Verification items for the finished model (mm, model axes). A direction names the side the tool comes from. Give positions to 0.01 mm unless a question says otherwise; leave off trailing zeros. Write each loop counter-clockwise with the first axis right and the second up, starting at its lowest first coordinate (ties: lowest second). Pieces come first, ordered by that corner, then holes. Notation, with made-up numbers: (39.25, 82.5) - (90.25, 82.5) arc R16 ccw to (90.25, 87.5) - close; hole circle Ø9 at (23.25, -24). An arc over 180 degrees is marked (long way). Answer as a JSON object with one key per item and string values. Group by question number.
Item 1: Scan lines: line 1 along X through (y, z) = (20, 0); line 2 along X through (y, z) = (37.5, -1); line 3 along Z through (x, y) = (70, 28.5). Record each from-to range of solid material in increasing order. Write a range as [from, to].
Item 2: Sectioned sample at B-B, the plane z = 0. Record the boundary of the cut face in (x, y).
Item 3: Sectioned sample at D-D, the plane z = 143. Record the boundary of the cut face in (x, y), and give its area (3 significant figures).
Item 4: Tool access check on faces 1 (the face through (112.81, 27.54, 63.11)), 2 (the face through (31, 40, 52)), 3 (the face through (-2, 25, -122)), 4 (the face through (2, 30, -149)). Record the directions out of +Z, -Z, +X, -X, +Y, -Y that give a thin tool (end or side, any length) a straight path to the whole face; none if there is none.
Item 5: Sectioned sample at A-A, the plane x = 0. Record the boundary of the cut face in (y, z), and give its area (4 significant figures).
Item 6: Go/stop test with flat-tipped pins: pin 1 (7.5 mm diameter, centred on x = -17.5, z = -121, fed in from +Y); pin 2 (15 mm diameter, centred on x = 1.5, z = -147.5, fed in from +Y); pin 3 (2.5 mm diameter, centred on x = -54.5, y = 28.5, fed in from +Z); pin 4 (1 mm diameter, centred on x = -136.5, z = -75, fed in from -Y). Record where each tip stops, or that it passes through.
Item 7: Sectioned sample at C-C, the plane y = 9. Record the boundary of the cut face in (x, z), and give its area (3 significant figures).
Item 8: Draft check along X on faces 5 (the face through (129, 30, 72)), 6 (the face through (-42.594, 34.93, -55.55)), 7 (the face through (107, 25, 59)), 8 (the face through (-111.06, 27.54, 66.14)). Enter one of: +X half, -X half, draft (parallel to the pull), parting line (faces both ways), or undercut.
```python
from build123d import *

# Parameters (mm, degrees)
SKETCH1_R           = 180
SKETCH1_R_2         = 60
BOSS_EXTRUDE1_DEPTH = 30
SKETCH2_R           = 70
SKETCH2_R_2         = 60
BOSS_EXTRUDE2_DEPTH = 10
SKETCH4_W           = 387.286858061
SKETCH4_H           = 15
CUT_EXTRUDE2_DEPTH  = 5
CIRPATTERN1_COUNT   = 3


with BuildPart() as part:
    # Sketch1 → Boss-Extrude1 (new body)
    with BuildSketch(Plane(origin=(0, 0, 0), x_dir=(1, 0, 0), z_dir=(0, 1, 0))):
        with Locations(Location((0, 0, 0), (0, 0, 270))):
            Circle(SKETCH1_R)
        with Locations(Location((0, 0, 0), (0, 0, 270))):
            Circle(SKETCH1_R_2, mode=Mode.SUBTRACT)
    extrude(amount=BOSS_EXTRUDE1_DEPTH)

    # Sketch2 → Boss-Extrude2 (add)
    with BuildSketch(Plane(origin=(0, 30, 0), x_dir=(1, 0, 0), z_dir=(0, 1, 0))):
        with Locations(Location((0, 0, 0), (0, 0, 270))):
            Circle(SKETCH2_R)
        with Locations(Location((0, 0, 0), (0, 0, 270))):
            Circle(SKETCH2_R_2, mode=Mode.SUBTRACT)
    extrude(amount=BOSS_EXTRUDE2_DEPTH)

    # Sketch4 → Cut-Extrude2 (cut)
    with BuildSketch(Plane(origin=(0, 30, 0), x_dir=(1, 0, 0), z_dir=(0, 1, 0))):
        with Locations((7.031744629, 121.75)):
            Rectangle(SKETCH4_W, SKETCH4_H)
    cut_extrude2 = extrude(amount=-CUT_EXTRUDE2_DEPTH, mode=Mode.SUBTRACT)

    # CirPattern1: Cut-Extrude2 ×3 about axis
    cirpattern1_axis = Axis((0, 0, 0), (0, 1, 0))
    for i in range(1, CIRPATTERN1_COUNT):
        add(cut_extrude2.rotate(cirpattern1_axis, i * 360 / CIRPATTERN1_COUNT), mode=Mode.SUBTRACT)


solid = part.part
```
Geometry check:
{
 "1": {"line 1": "[-180, -60], [60, 180]", "line 2": "[-69.99, -59.99], [59.99, 69.99]", "line 3": "[-165.83, -129.25], [-114.25, 107.26], [137.26, 165.83]"},
 "2": {"outline": "(-180, 0) - (-60, 0) - (-60, 40) - (-70, 40) - (-70, 30) - (-131.92, 30) - (-131.92, 25) - (-149.25, 25) - (-149.25, 30) - (-180, 30) - close; (60, 0) - (180, 0) - (180, 30) - (149.25, 30) - (149.25, 25) - (131.92, 25) - (131.92, 30) - (70, 30) - (70, 40) - (60, 40) - close"},
 "3": {"outline": "(-109.32, 0) - (109.32, 0) - (109.32, 30) - (66.68, 30) - (66.68, 25) - (49.36, 25) - (49.36, 30) - (-49.36, 30) - (-49.36, 25) - (-66.68, 25) - (-66.68, 30) - (-109.32, 30) - close", "area": "6,390 mm^2"},
 "4": {"face 1": "+Y", "face 2": "+Z, -Z, +X, -X, +Y", "face 3": "+X, -X, +Y", "face 4": "-Z, +X, -X, +Y"},
 "5": {"outline": "(0, -180) - (30, -180) - (30, -129.25) - (25, -129.25) - (25, -114.25) - (30, -114.25) - (30, -70) - (40, -70) - (40, -60) - (0, -60) - close; (0, 60) - (40, 60) - (40, 70) - (30, 70) - (30, 180) - (0, 180) - close", "area": "7,325 mm^2"},
 "6": {"pin 1": "y = 25", "pin 2": "y = 30", "pin 3": "z = 171.94", "pin 4": "y = 0"},
 "7": {"outline": "circle Ø360 at (0, 0); hole circle Ø120 at (0, 0)", "area": "90,500 mm^2"},
 "8": {"face 5": "draft", "face 6": "parting line", "face 7": "undercut", "face 8": "undercut"}
}
